Model file for the job. Use its own axes, mm. A direction names the side the tool comes from. Round coordinates to 2 decimals unless told otherwise and drop trailing zeros. Loops run counter-clockwise (first coordinate to the right, second up) from the corner with the lowest first, then second, coordinate; pieces in that order, holes last. Notation, with made-up numbers: M 19.25,50.25 L 30.25,50.25 A33 cw 30.25,78.25 Z; hole C -1.75,-37.75 d5. An arc over 180 degrees is marked long. Use a Markdown table: item, result. Add a question column.
Item 1: Tool access for faces 1 (the cylindrical face through (224.782, 9.893, 97.465)), 2 (the cylindrical face through (-249.76, 10.99, 245.44)), 3 (the flat face through (205, 94, 95)): list every direction of +Z, -Z, +X, -X, +Y, -Y with a clear straight run to the whole face (end or side of a thin tool).
Item 2: Saw through at D-D on y = -93. Write the cut outline in (x, z), then the cut area to 3 significant figures.
Item 3: Saw through at C-C on z = 371. Write the cut outline in (x, y), then the cut area to 3 significant figures.
Item 4: Two-plate mould, pull along X, no slides. Class faces 4 (the cylindrical face through (-32.936, 250.847, 197.2)), 5 (the flat face through (-245, 57, 0)), 6 (the flat face through (205, 94, 100)): +X half, -X half, draft (parallel to the pull), parting line (faces both ways), or undercut.
Item 5: Pin check, flat tips, straight feed: P1, Ø5, axis at y = 98.5, z = 151.5, coming from the -X side; P2, Ø5, axis at x = -118.75, y = -205.68, coming from the +Z side; P3, Ø6, axis at y = -190, z = 203, coming from the +X side; P4, Ø1.5, axis at x = -152.5, y = 194, coming from the +Z side. Stop position of each tip, or through.
Item 6: Wall check: L1, parallel to Y at x = -118, z = 96; L2, parallel to Y at x = -118.75, z = 96.7; L3, parallel to Z at x = 12, y = 253. Give the ranges that are in metal, low to high. Write a range as from..to.
Item 7: Saw through at B-B on y = 136. Write the cut outline in (x, z).
```python
from build123d import *

# Parameters (mm, degrees)
SKETCH1_R                = 253
SKETCH1_R_2              = 250
BOSS_EXTRUDE1_DEPTH      = 400
BOSS_EXTRUDE2_START      = -95
SKETCH2_R                = 250
SKETCH2_R_2              = 225
BOSS_EXTRUDE2_DEPTH      = 5
SKETCH3_R                = 3
CUT_EXTRUDE1_DEPTH       = 20
CIRPATTERN1_COUNT        = 6
BOSS_EXTRUDE4_REACH      = 697.047
BOSS_EXTRUDE4_END_RADIUS = 253
SKETCH6_W                = 40
SKETCH6_H                = 20
CUT_EXTRUDE2_REACH       = 697.047
CUT_EXTRUDE2_END_RADIUS  = 250
SKETCH8_R                = 2.604926317
CUT_EXTRUDE3_START       = -5
SKETCH9_R                = 251.5
SKETCH9_R_2              = 250
CUT_EXTRUDE3_DEPTH       = 5


with BuildPart() as part:
    # Sketch1 → Boss-Extrude1 (new body)
    with BuildSketch(Plane.XY):
        Circle(SKETCH1_R)
        Circle(SKETCH1_R_2, mode=Mode.SUBTRACT)
    extrude(amount=BOSS_EXTRUDE1_DEPTH)

    # Sketch2 → Boss-Extrude2 (add)
    with BuildSketch(Plane(origin=(0, 0, 0), x_dir=(-1, 0, 0), z_dir=(0, 0, -1)).offset(BOSS_EXTRUDE2_START)):
        Circle(SKETCH2_R)
        Circle(SKETCH2_R_2, mode=Mode.SUBTRACT)
    extrude(amount=-BOSS_EXTRUDE2_DEPTH)

    # Sketch3 → Cut-Extrude1 (cut)
    with BuildSketch(Plane(origin=(0, 0, 95), x_dir=(-1, 0, 0), z_dir=(0, 0, -1))):
        with Locations((237.5, 0)):
            Circle(SKETCH3_R)
    cut_extrude1 = extrude(amount=-CUT_EXTRUDE1_DEPTH, mode=Mode.SUBTRACT)

    # CirPattern1: Cut-Extrude1 ×6 about axis
    cirpattern1_axis = Axis((0, 0, 0), (0, 0, 1))
    for i in range(1, CIRPATTERN1_COUNT):
        add(cut_extrude1.rotate(cirpattern1_axis, i * 360 / CIRPATTERN1_COUNT), mode=Mode.SUBTRACT)

    # Boss-Extrude4: up to this cylinder (the profile starts outside it)
    boss_extrude4_end = Plane(origin=(0, 0, 390), z_dir=(0, 0, -1)) * Cylinder(BOSS_EXTRUDE4_END_RADIUS, 1901.094, mode=Mode.PRIVATE)
    # Sketch6 → Boss-Extrude4 (add, up to the surface)
    with BuildSketch(Plane(origin=(0, 256, 0), x_dir=(1, 0, 0), z_dir=(0, 1, 0)), mode=Mode.PRIVATE) as boss_extrude4_sk1:
        with Locations((0, -390)):
            Rectangle(SKETCH6_W, SKETCH6_H)
    boss_extrude4_tool1 = extrude(boss_extrude4_sk1.sketch, amount=-BOSS_EXTRUDE4_REACH, mode=Mode.PRIVATE) - boss_extrude4_end
    add(boss_extrude4_tool1.solids().sort_by_distance((0, 256, 390))[0])

    # Cut-Extrude2: up to this cylinder (the profile starts outside it)
    cut_extrude2_end = Plane(origin=(0, 0, 390), z_dir=(0, 0, -1)) * Cylinder(CUT_EXTRUDE2_END_RADIUS, 1895.094, mode=Mode.PRIVATE)
    # Sketch8 → Cut-Extrude2 (cut, up to the surface)
    with BuildSketch(Plane(origin=(0, 256, 0), x_dir=(1, 0, 0), z_dir=(0, 1, 0)), mode=Mode.PRIVATE) as cut_extrude2_sk1:
        with Locations(Location((-12.5, -390, 0), (0, 0, 270))):
            Circle(SKETCH8_R)
    cut_extrude2_tool1 = extrude(cut_extrude2_sk1.sketch, amount=-CUT_EXTRUDE2_REACH, mode=Mode.PRIVATE) - cut_extrude2_end
    add(cut_extrude2_tool1.solids().sort_by_distance((-12.5, 256, 390))[0], mode=Mode.SUBTRACT)
    # Sketch8 → Cut-Extrude2 (cut, up to the surface)
    with BuildSketch(Plane(origin=(0, 256, 0), x_dir=(1, 0, 0), z_dir=(0, 1, 0)), mode=Mode.PRIVATE) as cut_extrude2_sk2:
        with Locations(Location((12.5, -390, 0), (0, 0, 270))):
            Circle(SKETCH8_R)
    cut_extrude2_tool2 = extrude(cut_extrude2_sk2.sketch, amount=-CUT_EXTRUDE2_REACH, mode=Mode.PRIVATE) - cut_extrude2_end
    add(cut_extrude2_tool2.solids().sort_by_distance((12.5, 256, 390))[0], mode=Mode.SUBTRACT)

    # Sketch9 → Cut-Extrude3 (cut)
    with BuildSketch(Plane.XY.offset(400).offset(CUT_EXTRUDE3_START)):
        Circle(SKETCH9_R)
        with Locations(Location((0, 0, 0), (0, 0, 180))):
            Circle(SKETCH9_R_2, mode=Mode.SUBTRACT)
    extrude(amount=CUT_EXTRUDE3_DEPTH, mode=Mode.SUBTRACT)


solid = part.part
```
Entries:
| question | item | result |
|---|---|---|
| 1 | face 1 | +Z, -Z |
| 1 | face 2 | +Z |
| 1 | face 3 | -Z |
| 2 | outline | M -235.29,0 L -232.06,0 L -232.06,95 L -204.88,95 L -204.88,100 L -232.06,100 L -232.06,395 L -233.67,395 L -233.67,400 L -235.29,400 Z; M 204.88,95 L 232.06,95 L 232.06,0 L 235.29,0 L 235.29,400 L 233.67,400 L 233.67,395 L 232.06,395 L 232.06,100 L 204.88,100 Z |
| 2 | area | 2,840 mm2 |
| 3 | outline | C 0,0 d506; hole C 0,0 d500 |
| 3 | area | 4,740 mm2 |
| 4 | face 4 | parting line |
| 4 | face 5 | draft |
| 4 | face 6 | undercut |
| 5 | P1 | x = -234.08 |
| 5 | P2 | through |
| 5 | P3 | x = 170.41 |
| 5 | P4 | z = 100 |
| 6 | L1 | -223.8..-208.59, -202.78..-191.58, 191.58..202.78, 208.59..223.8 |
| 6 | L2 | -223.4..-208.68, -202.68..-191.11, 191.11..202.68, 208.68..223.4 |
| 6 | L3 | 380..387.44, 392.56..400 |
| 7 | outline | M -213.34,0 L -209.77,0 L -209.77,95 L -179.25,95 L -179.25,100 L -209.77,100 L -209.77,395 L -211.56,395 L -211.56,400 L -213.34,400 Z; M 179.25,95 L 209.77,95 L 209.77,0 L 213.34,0 L 213.34,400 L 211.56,400 L 211.56,395 L 209.77,395 L 209.77,100 L 179.25,100 Z |
